Drawing for the job (mm, zero at the part's lowest x, y, z). A direction names the side the tool comes from. Round coordinates to 2 decimals unless told otherwise and drop trailing zeros. Loops run counter-clockwise (first coordinate to the right, second up) from the corner with the lowest first, then second, coordinate; pieces in that order, holes last. Notation, with made-up numbers: M 5,31.25 L 13,31.25 A20 cw 13,69.25 Z; hole C 23,-16.75 d5. An arc over 180 degrees is marked long. Use a Markdown table: item, result. Add a question column.
Q1. Pin check, flat tips, straight feed: pin 1 (1.6 mm diameter, centred on x = 29, y = 1, fed in from -Z); pin 2 (8 mm diameter, centred on y = 24, z = 5.5, fed in from -X); pin 3 (16 mm diameter, centred on x = 20, z = 20, fed in from -Y); pin 4 (8 mm diameter, centred on x = 71, z = 10.5, fed in from +Y). Stop position of each tip, or through.
Q2. Tool access for the marked faces 1, 2, 3, 4 and 5: list every direction of +Z, -Z, +X, -X, +Y, -Y with a clear straight run to the whole face (end or side of a thin tool).
Q3. Probe line 1 (Y direction, x = 50, z = 2.75); line 2 (Z direction, x = 20, y = 5); line 3 (X direction, y = 6.5, z = 24). List the from-to ranges inside material, lowest first. Write a range as from..to.
Q4. Cut at C-C (z = 6.5). Give the cut face in (x, y).
Q5. Cut at A-A (z = 20). Give the cut face in (x, y).
Q6. Mould opens along X. For the marked faces 6, 7 and 8 say: +X half, -X half, draft (parallel to the pull), parting line (faces both ways), or undercut.
Q7. Cut at D-D (x = 32). Give the cut face in (y, z).
Q8. Cut at B-B (x = 50). Give the cut face in (y, z), plus the area to 3 significant figures.
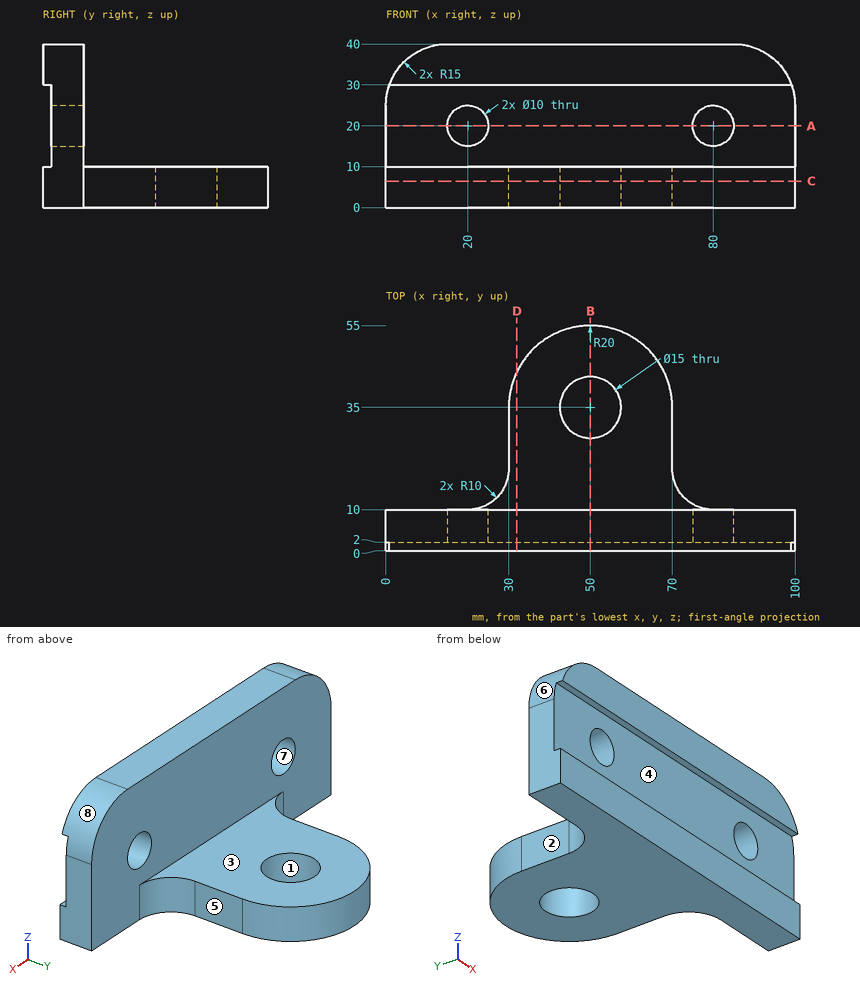
Checked values:
| question | item | result |
|---|---|---|
| 1 | pin 1 | stops at z = 0 |
| 1 | pin 2 | stops at x = 30 |
| 1 | pin 3 | stops at y = 2 |
| 1 | pin 4 | stops at y = 45.48 |
| 2 | face 1 | +Z, -Z |
| 2 | face 2 | +Z, -Z, -X, +Y |
| 2 | face 3 | +Z, +X, -X, +Y |
| 2 | face 4 | +X, -X, -Y |
| 2 | face 5 | +Z, -Z, +X, +Y |
| 3 | line 1 | y = 0..27.5, 42.5..55 |
| 3 | line 2 | z = 0..15, 25..40 |
| 3 | line 3 | x = 0..17, 23..77, 83..100 |
| 4 | outline | M 0,0 L 100,0 L 100,10 L 80,10 A10 cw 70,20 L 70,35 A20 ccw 30,35 L 30,20 A10 cw 20,10 L 0,10 Z; hole C 50,35 d15 |
| 5 | outline | M 0,2 L 15,2 L 15,10 L 0,10 Z; M 25,2 L 75,2 L 75,10 L 25,10 Z; M 85,2 L 100,2 L 100,10 L 85,10 Z |
| 6 | face 6 | -X half |
| 6 | face 7 | undercut |
| 6 | face 8 | +X half |
| 7 | outline | M 0,0 L 43.72,0 L 43.72,10 L 10,10 L 10,40 L 0,40 L 0,30 L 2,30 L 2,10 L 0,10 Z |
| 8 | outline | M 0,0 L 27.5,0 L 27.5,10 L 10,10 L 10,40 L 0,40 L 0,30 L 2,30 L 2,10 L 0,10 Z; M 42.5,0 L 55,0 L 55,10 L 42.5,10 Z |
| 8 | area | 660 mm^2 |
